from build123d import *

# Parameters (mm, degrees)
BOSS_EXTRUDE1_DEPTH     = 15
CHAMFER1_SIZE           = 1
SKETCH4_R               = 79.861717746
SKETCH4_R_2             = 50
CUT_EXTRUDE1_DEPTH      = 182.991758055
CUT_EXTRUDE2_DEPTH      = 195.321897891
CUT_EXTRUDE2_DEPTH_BACK = 195.321897891
SKETCH5_W               = 151.709550381
SKETCH5_H               = 33.031628388


with BuildPart() as part:
    # Sketch1 → Revolve1 (revolve)
    with BuildSketch(Plane.XY, mode=Mode.PRIVATE) as revolve1_sk:
        Polygon((35, 0), (60, 0), (60, 9.5), (59.5, 10), (60, 10.5), (60, 20), (42, 20), (21, 31), (15, 31), (15, 181), (0, 181), (0, 15), (14, 15), align=None)
    revolve(revolve1_sk.sketch.rotate(Axis((0, 181, 0), (0, -1, 0)), 180), axis=Axis((0, 181, 0), (0, -1, 0)))

    # Sketch2 → Boss-Extrude1 (add)
    with BuildSketch(Plane(origin=(0, 31, 0), x_dir=(1, 0, 0), z_dir=(0, 1, 0))):
        Polygon((15, 8.660254038), (0, 17.320508076), (-15, 8.660254038), (-15, -8.660254038), (0, -17.320508076), (15, -8.660254038), align=None)
    extrude(amount=BOSS_EXTRUDE1_DEPTH)

    # Sketch3 → Cut-Revolve1 (revolve, cut)
    with BuildSketch(Plane(origin=(0, 0, 0), x_dir=(0, 0, -1), z_dir=(1, 0, 0))):
        Polygon((15.820508076, 31), (17.320508076, 32.5), (17.320508076, 31), align=None)
        Polygon((17.320508076, 44.5), (15.820508076, 46), (17.320508076, 46), align=None)
    revolve(axis=Axis((0, 181, 0), (0, 1, 0)), mode=Mode.SUBTRACT)

    # Chamfer1
    chamfer1_edges = [part.edges().sort_by_distance(p)[0] for p in [
        (15, 181, 0),
    ]]
    chamfer(chamfer1_edges, length=CHAMFER1_SIZE)

    # Sketch4 → Cut-Extrude1 (cut, through all)
    with BuildSketch(Plane(origin=(0, 20, 0), x_dir=(1, 0, 0), z_dir=(0, 1, 0))):
        Circle(SKETCH4_R)
        with Locations(Location((0, 0, 0), (0, 0, 180))):
            Circle(SKETCH4_R_2, mode=Mode.SUBTRACT)
    extrude(amount=-CUT_EXTRUDE1_DEPTH, mode=Mode.SUBTRACT)

    # Sketch5 → Cut-Extrude2 (cut, two sides: drawn at the far end of the back side and taken through both)
    with BuildSketch(Plane.XY.offset(-CUT_EXTRUDE2_DEPTH_BACK)):
        with Locations((18.277609901, -6.515814194)):
            Rectangle(SKETCH5_W, SKETCH5_H)
    extrude(amount=CUT_EXTRUDE2_DEPTH + CUT_EXTRUDE2_DEPTH_BACK, mode=Mode.SUBTRACT)


solid = part.part
Here's how the part is built. I have some questions about the finished solid (model axes, mm). A direction names the side the tool comes from. Give positions to 0.01 mm unless a question says otherwise; leave off trailing zeros. Order: outer loops, then holes, each group sorted by start corner. A loop starts at its lowest first (then second) coordinate and runs counter-clockwise, first axis right, second up. Notation, with made-up numbers: (82, 30.25) -> (117, 30.25) arc R17 ccw to (117, 52.25) -> close; hole circle Ø4 at (45.25, 20). An arc over 180 degrees is marked (long way). One line per item, written item: value. Start each with the question number.
1. Imagine slicing it at A-A, the plane y = 147. List the corners of the cut face in (x, z) for me, plus the area to 3 significant figures.
2. For faces 4 (the face through (-15, 38, 0)), 5 (the face through (0, 15, 0)), 6 (the face through (-13.2, 46, -7.5)), 7 (the face through (15, 38, 0)), which set-ups out of +Z, -Z, +X, -X, +Y, -Y let a thin tool reach every point of the face, with its end or its side?
3. Imagine slicing it at B-B, the plane x = -44. List the corners of the cut face in (y, z) for me, plus the area to 3 significant figures.
4. I need wall thicknesses on probe 1 along Z at (x, y) = (-5.5, 146); probe 2 along X at (y, z) = (76, -1); probe 3 along X at (y, z) = (18, -36.5). Which ranges of each line are inside material? Lowest first, please. Write a range as from..to.
5. We'd pull the mould along Z, two halves only. Please class faces 1 (the face through (-13, 46, 8)), 2 (the face through (-8.06, 113.94, -12.65)), 3 (the face through (3.13, 14.69, 14.09)): released by +Z, released by -Z, zero draft, split by the parting line, or undercut.
6. Will these pins go through, and if not, where does the flat tip stop? pin 1 Ø8 at (x, z) = (-3, 29) entering from +Y; pin 2 Ø16.5 at (y, z) = (39, -3) entering from +X; pin 3 Ø0.8 at (x, z) = (-2, 14.5) entering from +Y.
Values follow:
1. outline: circle Ø30 at (0, 0)
1. area: 707 mm2
2. face 4: +Z, -Z, -X, +Y
2. face 5: -Y
2. face 6: -Z, -X, +Y
2. face 7: +Z, -Z, +X, +Y
3. outline: (10, -23.75) -> (20, -23.75) -> (20, 23.75) -> (10, 23.75) -> close
3. area: 475 mm2
4. probe 1: z = -13.96..13.96
4. probe 2: x = -14.97..14.97
4. probe 3: x = -34.17..34.17
5. face 1: zero draft
5. face 2: split by the parting line
5. face 3: undercut
6. pin 1: stops at y = 28.82
6. pin 2: stops at x = 21.3
6. pin 3: stops at y = 180.76
